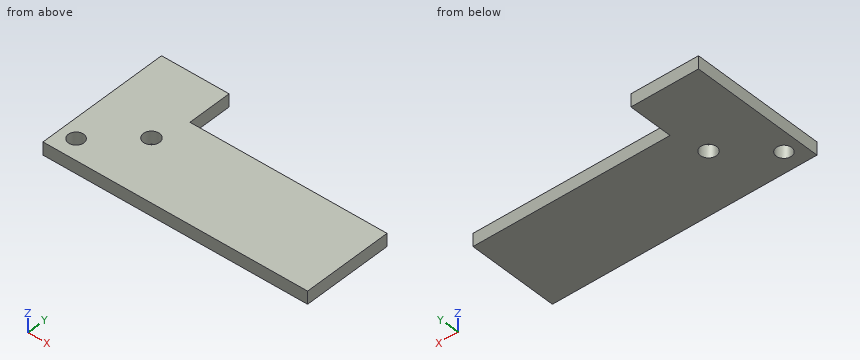
from build123d import *

# Parameters (mm, degrees)
SKETCH1_R           = 6
SKETCH1_R_2         = 6.25
BOSS_EXTRUDE1_DEPTH = 10


with BuildPart() as part:
    # Sketch1 → Boss-Extrude1 (new body)
    with BuildSketch(Plane.XY):
        Polygon((7.55, 34.5), (7.55, -70), (212.942105032, -70), (212.942105032, 0), (137.727272727, 0), (60, 0), (60, 34.5), align=None)
        with Locations((20, -55)):
            Circle(SKETCH1_R, mode=Mode.SUBTRACT)
        with Locations((52.55, -25.5)):
            Circle(SKETCH1_R_2, mode=Mode.SUBTRACT)
    extrude(amount=BOSS_EXTRUDE1_DEPTH)


solid = part.part
Work out the finished part from the listing and answer in its coordinate system (mm). Round coordinates to 2 decimals unless told otherwise and drop trailing zeros. Order: outer loops, then holes, each group sorted by start corner. A loop starts at its lowest first (then second) coordinate and runs counter-clockwise, first axis right, second up. Notation, with made-up numbers: M 69,18 L 103,18 A27 ccw 103,48 Z; hole C 79,-40 d3. An arc over 180 degrees is marked long. One line per item, written item: value.
Q1. Flat-ended cylindrical pins translate along their axes: pin 1 (3 mm diameter, centred on y = 17.5, z = 6.5, fed in from +X); pin 2 (11 mm diameter, centred on x = 52.55, y = -25.5, fed in from +Z); pin 3 (3 mm diameter, centred on x = 151, z = 5, fed in from +Y). Find the tip coordinate at first contact, or state that the pin passes through.
Derived:
pin 1: x = 60
pin 2: through
pin 3: y = 0
Q2. Find section D-D on y = 6. Write down the section's boundary in (x, z).
Derived:
outline: M 7.55,0 L 60,0 L 60,10 L 7.55,10 Z
Q3. Straight lines are drawn through the part: line 1 (Y direction, x = 52.55, z = 3); line 2 (Y direction, x = 20, z = 8); line 3 (X direction, y = 20, z = 4.75). For each, find the intervals that lie inside material, in ascending order.
Derived:
line 1: -70 to -31.75, -19.25 to 34.5
line 2: -70 to -61, -49 to 34.5
line 3: 7.55 to 60
Q4. Find section B-B on x = 20. Write down the section's boundary in (y, z).
Derived:
outline: M -70,0 L -61,0 L -61,10 L -70,10 Z; M -49,0 L 34.5,0 L 34.5,10 L -49,10 Z
Q5. Find section A-A on y = -25.5. Write down the section's boundary in (x, z), then the cut area to 3 significant figures.
Derived:
outline: M 7.55,0 L 46.3,0 L 46.3,10 L 7.55,10 Z; M 58.8,0 L 212.94,0 L 212.94,10 L 58.8,10 Z
area: 1,930 mm²
Q6. Find section C-C on z = 1.5. Write down the section's boundary in (x, y), then the cut area to 3 significant figures.
Derived:
outline: M 7.55,-70 L 212.94,-70 L 212.94,0 L 60,0 L 60,34.5 L 7.55,34.5 Z; hole C 20,-55 d12; hole C 52.55,-25.5 d12.5
area: 16,000 mm²
